Can you work these out from the model? Positions are in its coordinate system, mm. A direction names the side the tool comes from. Round coordinates to 2 decimals unless told otherwise and drop trailing zeros. Order: outer loops, then holes, each group sorted by start corner. A loop starts at its lowest first (then second) coordinate and runs counter-clockwise, first axis right, second up. Notation, with made-up numbers: (18.25, 26.25) -> (72.25, 26.25) arc R30 ccw to (72.25, 55.25) -> close; hole circle Ø10 at (84.25, -7). An arc over 180 degrees is marked (long way). Use a Markdown table: item, result. Add a question column.
Q1. If we section it at A-A on y = 22: List the corners of the cut face in (x, z) for me, plus the area to 3 significant figures.
Q2. If we section it at C-C on x = -6.25: List the corners of the cut face in (y, z) for me, plus the area to 3 significant figures.
Q3. For faces 1 (the face through (-10, 21, 9)), 2 (the face through (0, -1, 9)), which set-ups out of +Z, -Z, +X, -X, +Y, -Y let a thin tool reach every point of the face, with its end or its side?
Q4. If we section it at B-B on z = -541.5: List the corners of the cut face in (x, y) for me, plus the area to 3 significant figures.
Q5. I need wall thicknesses on line 1 along Y through (x, z) = (-7, 98); line 2 along Y through (x, z) = (-2.5, -239.5); line 3 along X through (y, z) = (23, 20.5). Which ranges of each line are inside material? Lowest first, please. Write a range as [from, to].
Q6. We'd pull the mould along Y, two halves only. Please class faces 3 (the face through (-12, 21, 9)), 4 (the face through (-2, -22, 9)): +Y half, -Y half, draft (parallel to the pull), parting line (faces both ways), or undercut.
```python
from build123d import *

# Parameters (mm, degrees)
SKETCH_1_W      = 8
SKETCH_1_H      = 26
EXTRUDE_1_DEPTH = 625


with BuildPart() as part:
    # 草图1 → 凸台-拉伸1 (new, symmetric)
    with BuildSketch(Plane.XY):
        Polygon((-12, 4.5), (-10, 4.5), (-10, 6.5), (-4, 6.5), (-4, -6.5), (-10, -6.5), (-10, -4.5), (-12, -4.5), (-12, -36.5), (0, -36.5), (0, 36.5), (-12, 36.5), align=None)
        with Locations((-6, -21.5)):
            Rectangle(SKETCH_1_W, SKETCH_1_H, mode=Mode.SUBTRACT)
        with Locations((-6, 21.5)):
            Rectangle(SKETCH_1_W, SKETCH_1_H, mode=Mode.SUBTRACT)
    extrude(amount=EXTRUDE_1_DEPTH, both=True)


solid = part.part
```
Answer below:
| question | item | result |
|---|---|---|
| 1 | outline | (-12, -625) -> (-10, -625) -> (-10, 625) -> (-12, 625) -> close; (-2, -625) -> (0, -625) -> (0, 625) -> (-2, 625) -> close |
| 1 | area | 5,000 mm² |
| 2 | outline | (-36.5, -625) -> (-34.5, -625) -> (-34.5, 625) -> (-36.5, 625) -> close; (-8.5, -625) -> (-6.5, -625) -> (-6.5, 625) -> (-8.5, 625) -> close; (6.5, -625) -> (8.5, -625) -> (8.5, 625) -> (6.5, 625) -> close; (34.5, -625) -> (36.5, -625) -> (36.5, 625) -> (34.5, 625) -> close |
| 2 | area | 10,000 mm² |
| 3 | face 1 | +Z, -Z |
| 3 | face 2 | +Z, -Z, +X, +Y, -Y |
| 4 | outline | (-12, -36.5) -> (0, -36.5) -> (0, 36.5) -> (-12, 36.5) -> (-12, 4.5) -> (-10, 4.5) -> (-10, 6.5) -> (-4, 6.5) -> (-4, -6.5) -> (-10, -6.5) -> (-10, -4.5) -> (-12, -4.5) -> close; hole (-10, -34.5) -> (-2, -34.5) -> (-2, -8.5) -> (-10, -8.5) -> close; hole (-10, 8.5) -> (-2, 8.5) -> (-2, 34.5) -> (-10, 34.5) -> close |
| 4 | area | 364 mm² |
| 5 | line 1 | [-36.5, -34.5], [-8.5, -6.5], [6.5, 8.5], [34.5, 36.5] |
| 5 | line 2 | [-36.5, -34.5], [-8.5, 8.5], [34.5, 36.5] |
| 5 | line 3 | [-12, -10], [-2, 0] |
| 6 | face 3 | draft |
| 6 | face 4 | undercut |
